```python
from build123d import *

# Parameters (mm, degrees)
LINK_PROFILE_SKETCH_R    = 9
LINK_BODY_DEPTH          = 20.5
EYE_RECESS_CUT_5MM_DEPTH = 5
SLOT_SKETCH_W            = 14
SLOT_SKETCH_H            = 12
SLOT_CUT_14X12_DEPTH     = 75
END_CHAMFER_3MM_SIZE     = 3


with BuildPart() as part:
    # Link Profile Sketch → Link Body (new, symmetric)
    with BuildSketch(Plane(origin=(0, 0, 0), x_dir=(1, 0, 0), z_dir=(0, 1, 0))):
        with BuildLine():
            Line((9.704358302, -32), (54.704358302, -32))
            Line((54.704358302, -32), (54.704358302, 0))
            Line((54.704358302, 0), (9.704358302, 0))
            Line((9.704358302, 0), (-5, 21))
            Line((-5, 21), (-55, 21))
            ThreePointArc((-55, 21), (-76, 0), (-55, -21))
            Line((-55, -21), (-0.295641698, -21))
            ThreePointArc((-0.295641698, -21), (6.775426114, -23.928932188), (9.704358302, -31))
            Line((9.704358302, -31), (9.704358302, -32))
        make_face()
        with Locations(Location((-55, 0, 0), (0, 0, 270))):
            Circle(LINK_PROFILE_SKETCH_R, mode=Mode.SUBTRACT)
    extrude(amount=LINK_BODY_DEPTH, both=True)

    # Eye Recess Sketch → Eye Recess Cut 5mm (cut)
    with BuildSketch(Plane(origin=(0, 20.5, 0), x_dir=(1, 0, 0), z_dir=(0, 1, 0))):
        with BuildLine():
            Line((-55, -21), (-34, -21))
            Line((-34, -21), (-34, 21))
            Line((-34, 21), (-55, 21))
            ThreePointArc((-55, 21), (-76, 0), (-55, -21))
        make_face()
    extrude(amount=-EYE_RECESS_CUT_5MM_DEPTH, mode=Mode.SUBTRACT)

    # Slot Sketch → Slot Cut 14x12 (cut)
    with BuildSketch(Plane(origin=(54.704358302, 0, 0), x_dir=(0, 0, -1), z_dir=(1, 0, 0))):
        with Locations((-32, 0)):
            Rectangle(SLOT_SKETCH_W, SLOT_SKETCH_H)
    extrude(amount=-SLOT_CUT_14X12_DEPTH, mode=Mode.SUBTRACT)

    # End Chamfer 3mm
    end_chamfer_3mm_edges = [part.edges().sort_by_distance(p)[0] for p in [
        (54.704358302, -20.5, 16),
        (-19.5, 20.5, -21),
        (54.704358302, 20.5, 16),
    ]]
    chamfer(end_chamfer_3mm_edges, length=END_CHAMFER_3MM_SIZE)


solid = part.part
```
The model under review builds one solid part; all positions refer to its coordinate system, in mm. A direction names the side the tool comes from. Give positions to 0.01 mm unless a question says otherwise; leave off trailing zeros. Write each loop counter-clockwise with the first axis right and the second up, starting at its lowest first coordinate (ties: lowest second). Pieces come first, ordered by that corner, then holes. Notation, with made-up numbers: (77.5, -6) - (98.5, -6) arc R29 cw to (98.5, 21) - close; hole circle Ø8 at (28.25, -25). An arc over 180 degrees is marked (long way). Answer in a Markdown table with one row per item. Add a question column.
1. We need section A-A on y = -12.5. Write out the cut boundary in (x, z).
2. Draft analysis for pull direction Y (two halves, no side actions). For faces 1 (the flat face through (-46, 15.5, 4)), 2 (the flat face through (32, -13, 32)), 3 (the flat face through (32, 6, 29)), state which applies: +Y half, -Y half, draft (parallel to the pull), parting line (faces both ways), or undercut.
3. We need section C-C on x = 42.5. Write out the cut boundary in (y, z), then the cut area to 3 significant figures.
4. We need section B-B on x = -62.5. Write out the cut boundary in (y, z).
5. Insertion check: P1, Ø20.5, axis at x = 37.5, y = -0.5, coming from the -Z side; P2, Ø21, axis at x = -56.5, z = 0, coming from the +Y side; P3, Ø1.5, axis at y = 19, z = 2.5, coming from the -X side. Each pin has a flat end and moves straight along its axis. Give the tip position at first contact, or say it passes through.
6. Tool access review of faces 4 (the flat face through (-28, 0, 21)), 5 (the flat face through (32, -6, 29)), 6 (the flat face through (-34, 18, 0)), 7 (the flat face through (-13, -20.5, 5)): name each direction out of +Z, -Z, +X, -X, +Y, -Y from which nothing blocks a thin tool from reaching the whole face with its end or side.
7. We need section D-D on z = 22.5. Write out the cut boundary in (x, y), then the cut area to 3 significant figures.
8. Wall thickness on line 1 along Z through (x, y) = (-55, -1); line 2 along Y through (x, z) = (45.5, 30); line 3 along Y through (x, z) = (-38, 14): over which ranges is each line inside the solid? List them lowest first. Write a range as [from, to].
Ans:
| question | item | result |
|---|---|---|
| 1 | outline | (-55, -21) - (-5, -21) - (9.7, 0) - (54.7, 0) - (54.7, 32) - (9.7, 32) - (9.7, 31) arc R10 cw to (-0.3, 21) - (-55, 21) arc R21 ccw to start; hole circle Ø18 at (-55, 0) |
| 2 | face 1 | +Y half |
| 2 | face 2 | draft |
| 2 | face 3 | undercut |
| 3 | outline | (-20.5, 0) - (20.5, 0) - (20.5, 32) - (6, 32) - (6, 25) - (-6, 25) - (-6, 32) - (-20.5, 32) - close |
| 3 | area | 1,230 mm^2 |
| 4 | outline | (-20.5, -19.62) - (15.5, -19.62) - (15.5, -4.97) - (-20.5, -4.97) - close; (-20.5, 4.97) - (15.5, 4.97) - (15.5, 19.62) - (-20.5, 19.62) - close |
| 5 | P1 | stops at z = 0 |
| 5 | P2 | stops at y = 15.5 |
| 5 | P3 | stops at x = -34 |
| 6 | face 4 | +Z, -X, +Y, -Y |
| 6 | face 5 | +Z, +X, -X |
| 6 | face 6 | +Z, -Z, -X, +Y |
| 6 | face 7 | +Z, -Z, +X, -X, -Y |
| 7 | outline | (4.97, -20.5) - (51.7, -20.5) - (54.7, -17.5) - (54.7, 17.5) - (51.7, 20.5) - (4.97, 20.5) - close |
| 7 | area | 2,030 mm^2 |
| 8 | line 1 | z = [-21, -9], [9, 21] |
| 8 | line 2 | y = [-20.5, -6], [6, 20.5] |
| 8 | line 3 | y = [-20.5, 15.5] |
